Model file for the job. Use its own axes, mm. A direction names the side the tool comes from. Round coordinates to 2 decimals unless told otherwise and drop trailing zeros. Order: outer loops, then holes, each group sorted by start corner. A loop starts at its lowest first (then second) coordinate and runs counter-clockwise, first axis right, second up. Notation, with made-up numbers: (72.5, 21.5) -> (80.5, 21.5) arc R20 ccw to (80.5, 44.5) -> close; hole circle Ø4 at (0, 29). An arc over 180 degrees is marked (long way). Use CSV: the item, a comma, the result in double quotes.
```python
from build123d import *

# Parameters (mm, degrees)
SKETCH1_R             = 12.5
BOSS_EXTRUDE1_DEPTH   = 243
SKETCH2_W             = 20
SKETCH2_H             = 15
CUT_EXTRUDE1_DEPTH    = 68
M6_TAPPED_HOLE1_D     = 5
M6_TAPPED_HOLE1_DEPTH = 15
M6_TAPPED_HOLE1_TIP   = 1.502151548
M6_TAPPED_HOLE2_D     = 5
M6_TAPPED_HOLE2_DEPTH = 15
M6_TAPPED_HOLE2_TIP   = 1.502151548
SKETCH7_W             = 2.5
SKETCH7_H             = 15
CUT_EXTRUDE2_DEPTH    = 160
M4_TAPPED_HOLE1_D     = 3.3
M4_TAPPED_HOLE1_DEPTH = 10.1
M4_TAPPED_HOLE1_TIP   = 0.991420021
SKETCH10_R            = 3
CUT_EXTRUDE3_DEPTH    = 10
CHAMFER1_SIZE         = 1


with BuildPart() as part:
    # Sketch1 → Boss-Extrude1 (new body)
    with BuildSketch(Plane.XY):
        Circle(SKETCH1_R)
    extrude(amount=BOSS_EXTRUDE1_DEPTH)

    # Sketch2 → Cut-Extrude1 (cut)
    with BuildSketch(Plane.XY):
        with Locations((20, 0)):
            Rectangle(SKETCH2_W, SKETCH2_H)
    extrude(amount=CUT_EXTRUDE1_DEPTH, mode=Mode.SUBTRACT)

    # M6 Tapped Hole1
    with Locations(Plane.XY.offset(243)):
        with Locations((0, 0)):
            Hole(M6_TAPPED_HOLE1_D / 2, depth=M6_TAPPED_HOLE1_DEPTH)
            with Locations((0, 0, -(M6_TAPPED_HOLE1_DEPTH + M6_TAPPED_HOLE1_TIP / 2))):  # 118° drill point
                Cone(0, M6_TAPPED_HOLE1_D / 2, M6_TAPPED_HOLE1_TIP, mode=Mode.SUBTRACT)

    # M6 Tapped Hole2
    with Locations(Plane(origin=(10, 0, 0), x_dir=(0, 0, -1), z_dir=(1, 0, 0))):
        with Locations((-13, 0), (-53, 0)):
            Hole(M6_TAPPED_HOLE2_D / 2, depth=M6_TAPPED_HOLE2_DEPTH)
            with Locations((0, 0, -(M6_TAPPED_HOLE2_DEPTH + M6_TAPPED_HOLE2_TIP / 2))):  # 118° drill point
                Cone(0, M6_TAPPED_HOLE2_D / 2, M6_TAPPED_HOLE2_TIP, mode=Mode.SUBTRACT)

    # Sketch7 → Cut-Extrude2 (cut)
    with BuildSketch(Plane(origin=(0, 0, 0), x_dir=(-1, 0, 0), z_dir=(0, 0, -1))):
        with Locations((11.25, 0)):
            Rectangle(SKETCH7_W, SKETCH7_H)
    extrude(amount=-CUT_EXTRUDE2_DEPTH, mode=Mode.SUBTRACT)

    # M4 Tapped Hole1
    with Locations(Plane.ZY.offset(10)):
        with Locations((8, 0), (83, 0), (48, 0)):
            Hole(M4_TAPPED_HOLE1_D / 2, depth=M4_TAPPED_HOLE1_DEPTH)
            with Locations((0, 0, -(M4_TAPPED_HOLE1_DEPTH + M4_TAPPED_HOLE1_TIP / 2))):  # 118° drill point
                Cone(0, M4_TAPPED_HOLE1_D / 2, M4_TAPPED_HOLE1_TIP, mode=Mode.SUBTRACT)

    # Sketch10 → Cut-Extrude3 (cut)
    with BuildSketch(Plane(origin=(10, 0, 0), x_dir=(0, 0, -1), z_dir=(1, 0, 0))):
        with Locations((-33, 0)):
            Circle(SKETCH10_R)
    extrude(amount=-CUT_EXTRUDE3_DEPTH, mode=Mode.SUBTRACT)

    # Chamfer1
    chamfer1_edges = [part.edges().sort_by_distance(p)[0] for p in [
        (0, 12.5, 0),
        (0, -12.5, 0),
        (-12.5, 0, 243),
    ]]
    chamfer(chamfer1_edges, length=CHAMFER1_SIZE)


solid = part.part
```
Q1. Cut at A-A (z = 169.5). Give the cut face in (x, y).
From the geometry:
outline,"circle Ø25 at (0, 0)"
Q2. Mould opens along Z. For faces 6 (the cylindrical face through (5, 0, 36)), 7 (the cylindrical face through (0.54, -2.44, 235.4)), 8 (the flat face through (0, 0, 0)), 9 (the flat face through (0, 0, 33)) say: +Z half, -Z half, draft (parallel to the pull), parting line (faces both ways), or undercut.
From the geometry:
face 6,"undercut"
face 7,"draft"
face 8,"-Z half"
face 9,"undercut"
Q3. Cut at C-C (z = 65). Give the cut face in (x, y).
From the geometry:
outline,"(-10, -7.5) arc R12.5 ccw to (10, -7.5) -> (10, 7.5) arc R12.5 ccw to (-10, 7.5) -> close"
Q4. Cut at B-B (z = 134). Give the cut face in (x, y), plus the area to 3 significant figures.
From the geometry:
outline,"(-10, -7.5) arc R12.5 ccw (long way) to (-10, 7.5) -> close"
area,"465 mm²"
Q5. Pin check, flat tips, straight feed: pin 1 (12 mm diameter, centred on x = 7.5, z = 212, fed in from +Y); pin 2 (7 mm diameter, centred on y = 0, z = 33, fed in from +X); pin 3 (1 mm diameter, centred on x = 8, z = 143.5, fed in from -Y). Stop position of each tip, or through.
From the geometry:
pin 1,"stops at y = 12.41"
pin 2,"stops at x = 10"
pin 3,"stops at y = -10"
Q6. Probe line 1 along Z through (x, y) = (3.75, -0.25); line 2 along Z through (x, y) = (-3, 0); line 3 along Z through (x, y) = (-6.75, 0). List the from-to ranges inside material, lowest first.
From the geometry:
line 1,"z = 0 to 10.51, 15.49 to 30.01, 35.99 to 50.51, 55.49 to 243"
line 2,"z = 0 to 6.35, 9.65 to 10.5, 15.5 to 46.35, 49.65 to 50.5, 55.5 to 81.35, 84.65 to 243"
line 3,"z = 0 to 6.35, 9.65 to 46.35, 49.65 to 81.35, 84.65 to 243"
Q7. Which spindle directions (+Z, -Z, +X, -X, +Y, -Y) get a long thin tool onto all of the face, cutting with end or side? Do faces 1 (the flat face through (-10, 0, 79)), 2 (the flat face through (10, 3, 34)), 3 (the cylindrical face through (2.4, 0.1, 10.5)), 4 (the flat face through (-3, 0, 243)), 5 (the conical face through (-0.2, -11.7, 0.2)). Say none if no direction does.
From the geometry:
face 1,"-Z, -X, +Y, -Y"
face 2,"-Z, +X, +Y, -Y"
face 3,"+X"
face 4,"+Z, +X, -X, +Y, -Y"
face 5,"-Z, -Y"
